The listing builds one solid part. Answer for the finished solid, in the listing's coordinates (mm). Face numbers are marked on the shaded views. Give positions to 0.01 mm unless a question says otherwise; leave off trailing zeros. Write each loop counter-clockwise with the first axis right and the second up, starting at its lowest first coordinate (ties: lowest second). Pieces come first, ordered by that corner, then holes.
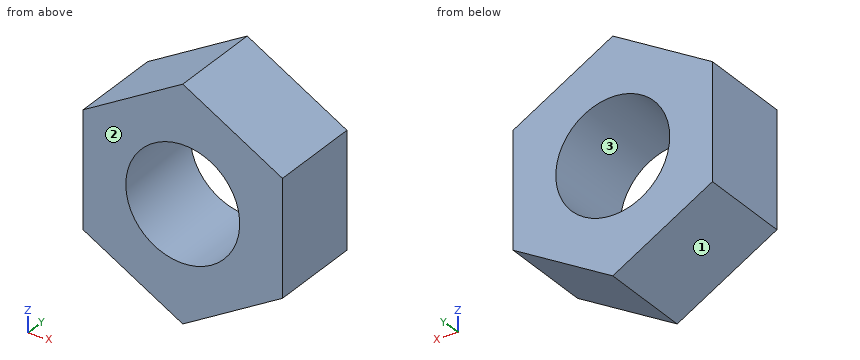
```python
from build123d import *

# Parameters (mm, degrees)
EXTRUDE_1_DEPTH     = 10
HOLE_WIZARD_M14_1_D = 12


with BuildPart() as part:
    # 草图1 → 凸台-拉伸1 (new body)
    with BuildSketch(Plane(origin=(0, 0, 0), x_dir=(1, 0, 0), z_dir=(0, 1, 0))):
        Polygon((0, 12.124355653), (-10.5, 6.062177826), (-10.5, -6.062177826), (0, -12.124355653), (10.5, -6.062177826), (10.5, 6.062177826), align=None)
    extrude(amount=EXTRUDE_1_DEPTH)

    # M14 螺纹孔1 (through all)
    with Locations(Plane(origin=(0, 10, 0), x_dir=(1, 0, 0), z_dir=(0, 1, 0))):
        with Locations((0, 0)):
            Hole(HOLE_WIZARD_M14_1_D / 2)


solid = part.part
```
Item 1: A cutting plane is placed at A-A, the plane z = 0. Give the vertices of the cut face in (x, y).
Conclusion:
outline: (-10.5, 0) - (-6, 0) - (-6, 10) - (-10.5, 10) - close; (6, 0) - (10.5, 0) - (10.5, 10) - (6, 10) - close
Item 2: A cutting plane is placed at B-B, the plane y = 2.25. Give the vertices of the cut face in (x, z).
Conclusion:
outline: (-10.5, -6.06) - (0, -12.12) - (10.5, -6.06) - (10.5, 6.06) - (0, 12.12) - (-10.5, 6.06) - close; hole circle Ø12 at (0, 0)
Item 3: Determine the mould class of the marked faces 1, 2 and 3 for opening direction X: pulls with the +X half, pulls with the -X half, needs draft (parallel to the pull), parting line crosses it, or undercut.
Conclusion:
face 1: pulls with the -X half
face 2: needs draft
face 3: undercut
Item 4: A cutting plane is placed at C-C, the plane x = -1.5. Give the vertices of the cut face in (y, z).
Conclusion:
outline: (0, -11.26) - (10, -11.26) - (10, -5.81) - (0, -5.81) - close; (0, 5.81) - (10, 5.81) - (10, 11.26) - (0, 11.26) - close
Item 5: This flat-tipped pin is pushed along its axis until it touches: P1, Ø5, axis at x = -1, z = -3, coming from the -Y side. Where does it stop, or does it pass through?
Conclusion:
P1: passes through
Item 6: Consider probe 1 along X at (y, z) = (5, 3.75); probe 2 along Z at (x, y) = (0.5, 2.25); probe 3 along Z at (x, y) = (3.25, 2.5). Determine where each line is inside the solid, lowest interval first.
Conclusion:
probe 1: x = -10.5 to -4.68, 4.68 to 10.5
probe 2: z = -11.84 to -5.98, 5.98 to 11.84
probe 3: z = -10.25 to -5.04, 5.04 to 10.25
